Geometry check sheet. Reference: the model listing, model coordinates, mm. A direction names the side the tool comes from. Round coordinates to 2 decimals unless told otherwise and drop trailing zeros. Order: outer loops, then holes, each group sorted by start corner. A loop starts at its lowest first (then second) coordinate and runs counter-clockwise, first axis right, second up.
```python
from build123d import *

# Parameters (mm, degrees)
SKETCH1_R           = 5.5
BOSS_EXTRUDE1_DEPTH = 40
SKETCH2_R           = 9
BOSS_EXTRUDE2_DEPTH = 12
CUT_EXTRUDE1_DEPTH  = 6


with BuildPart() as part:
    # Sketch1 → Boss-Extrude1 (new body)
    with BuildSketch(Plane.XY):
        Circle(SKETCH1_R)
    extrude(amount=BOSS_EXTRUDE1_DEPTH)

    # Sketch2 → Boss-Extrude2 (add)
    with BuildSketch(Plane.XY.offset(40)):
        Circle(SKETCH2_R)
    extrude(amount=BOSS_EXTRUDE2_DEPTH)

    # Sketch3 → Cut-Extrude1 (cut)
    with BuildSketch(Plane.XY.offset(52)):
        Polygon((0, 5.773502692), (-5, 2.886751346), (-5, -2.886751346), (0, -5.773502692), (5, -2.886751346), (5, 2.886751346), align=None)
    extrude(amount=-CUT_EXTRUDE1_DEPTH, mode=Mode.SUBTRACT)


solid = part.part
```
(1) Sectioned sample at B-B, the plane y = 0. Record the cut outline in (x, z), and give its area (3 significant figures).
Returned:
outline: (-9, 40) - (-5.5, 40) - (-5.5, 0) - (5.5, 0) - (5.5, 40) - (9, 40) - (9, 52) - (5, 52) - (5, 46) - (-5, 46) - (-5, 52) - (-9, 52) - close
area: 596 mm2
(2) Sectioned sample at A-A, the plane z = 47. Record the cut outline in (x, y).
Returned:
outline: circle Ø18 at (0, 0); hole (-5, -2.89) - (0, -5.77) - (5, -2.89) - (5, 2.89) - (0, 5.77) - (-5, 2.89) - close
(3) Material ranges on line 1 (Z direction, x = -4.75, y = -6); line 2 (Z direction, x = -1.5, y = -0.25); line 3 (X direction, y = -4, z = 25), recorded low to high.
Returned:
line 1: z = 40 to 52
line 2: z = 0 to 46
line 3: x = -3.77 to 3.77
(4) Sectioned sample at D-D, the plane x = 7.25. Record the cut outline in (y, z), and give its area (3 significant figures).
Returned:
outline: (-5.33, 40) - (5.33, 40) - (5.33, 52) - (-5.33, 52) - close
area: 128 mm2
(5) Depth check by flat-ended pin: P1, Ø3, axis at y = 0.5, z = 30, coming from the -X side; P2, Ø4, axis at y = -5, z = 47, coming from the +X side; P3, Ø1, axis at x = -1.5, z = 28.5, coming from the -Y side. Enter the tip coordinate at first touch or a pass-through.
Returned:
P1: stops at x = -5.5
P2: stops at x = 8.49
P3: stops at y = -5.41
(6) Draft check along Y on faces 4 (the flat face through (-4, -4, 40)), 5 (the cylindrical face through (-1.172, 8.923, 45.916)), 6 (the flat face through (2.465, -4.35, 49.042)). Enter one of: released by +Y, released by -Y, zero draft, split by the parting line, or undercut.
Returned:
face 4: zero draft
face 5: split by the parting line
face 6: undercut
(7) Set-up check for faces 1 (the flat face through (0, 0, 0)), 2 (the flat face through (-2.535, -4.31, 49.042)), 3 (the cylindrical face through (-1.19, -5.37, 19.72)): record each of +Z, -Z, +X, -X, +Y, -Y from which the full face is reachable in a straight line by a thin tool's end or side.
Returned:
face 1: -Z, +X, -X, +Y, -Y
face 2: +Z
face 3: -Z
(8) Sectioned sample at C-C, the plane z = 36.5. Record the cut outline in (x, y).
Returned:
outline: circle Ø11 at (0, 0)
